Could you check a few things on this model? Use its own coordinates, in mm. Give positions to 0.01 mm unless a question says otherwise; leave off trailing zeros. Write each loop counter-clockwise with the first axis right and the second up, starting at its lowest first coordinate (ties: lowest second). Pieces come first, ordered by that corner, then holes. Notation, with made-up numbers: (23, -23.5) - (59, -23.5) arc R7 ccw to (59, -17.5) - close; hole circle Ø2 at (16, 14). An arc over 180 degrees is marked (long way). Answer in a Markdown table with one row per item.
from build123d import *

# Parameters (mm, degrees)
SKETCH_1_W          = 190
SKETCH_1_H          = 28
EXTRUDE_1_DEPTH     = 10
SKETCH_2_R          = 3.5
SKETCH_2_R_2        = 10
CUT_EXTRUDE_1_DEPTH = 846.854305824


with BuildPart() as part:
    # 草图1 → 凸台-拉伸1 (new body)
    with BuildSketch(Plane(origin=(0, 1805.000303929, 0), x_dir=(1, 0, 0), z_dir=(0, 1, 0))):
        with Locations((602.085724054, 465)):
            Rectangle(SKETCH_1_W, SKETCH_1_H)
    extrude(amount=EXTRUDE_1_DEPTH)

    # 草图2 → 切除-拉伸1 (cut, through all)
    with BuildSketch(Plane(origin=(0, 1815.000303929, 0), x_dir=(1, 0, 0), z_dir=(0, 1, 0))):
        with Locations(Location((532.085724054, 465, 0), (0, 0, 180))):
            Circle(SKETCH_2_R)
        with Locations(Location((672.085724054, 465, 0), (0, 0, 180))):
            Circle(SKETCH_2_R)
        with Locations(Location((602.085724054, 465, 0), (0, 0, 180))):
            Circle(SKETCH_2_R_2)
    extrude(amount=-CUT_EXTRUDE_1_DEPTH, mode=Mode.SUBTRACT)


solid = part.part
1) We'd pull the mould along X, two halves only. Please class faces 1 (the face through (601, 1810, -479)), 2 (the face through (674.863, 1810.07, -467.13)), 3 (the face through (507.086, 1810, -465)): +X half, -X half, draft (parallel to the pull), parting line (faces both ways), or undercut.
Check values:
| item | result |
|---|---|
| face 1 | draft |
| face 2 | undercut |
| face 3 | -X half |
2) Imagine slicing it at B-B (y = 1810.25). List the corners of the cut face in (x, z) for me.
Check values:
| item | result |
|---|---|
| outline | (507.09, -479) - (697.09, -479) - (697.09, -451) - (507.09, -451) - close; hole circle Ø7 at (532.09, -465); hole circle Ø20 at (602.09, -465); hole circle Ø7 at (672.09, -465) |
3) Imagine slicing it at A-A (z = -465). List the corners of the cut face in (x, y) for me.
Check values:
| item | result |
|---|---|
| outline | (507.09, 1805) - (528.59, 1805) - (528.59, 1815) - (507.09, 1815) - close; (535.59, 1805) - (592.09, 1805) - (592.09, 1815) - (535.59, 1815) - close; (612.09, 1805) - (668.59, 1805) - (668.59, 1815) - (612.09, 1815) - close; (675.59, 1805) - (697.09, 1805) - (697.09, 1815) - (675.59, 1815) - close |
4) If I drill on line 1 (X direction, y = 1810.5, z = -464.75); line 2 (X direction, y = 1807.5, z = -465.75); line 3 (X direction, y = 1808, z = -471.75), over which ranges is the centre line in solid material (lowest first)?
Check values:
| item | result |
|---|---|
| line 1 | x = 507.09 to 528.59, 535.58 to 592.09, 612.08 to 668.59, 675.58 to 697.09 |
| line 2 | x = 507.09 to 528.67, 535.5 to 592.11, 612.06 to 668.67, 675.5 to 697.09 |
| line 3 | x = 507.09 to 594.71, 609.46 to 697.09 |
5) Imagine slicing it at C-C (x = 530.5). List the corners of the cut face in (y, z) for me.
Check values:
| item | result |
|---|---|
| outline | (1805, -479) - (1815, -479) - (1815, -468.12) - (1805, -468.12) - close; (1805, -461.88) - (1815, -461.88) - (1815, -451) - (1805, -451) - close |
6) Will this pin go through, and if not, where does the flat tip stop? P1, Ø4, axis at x = 532.09, z = -465, coming from the +Y side.
Check values:
| item | result |
|---|---|
| P1 | passes through |
